```python
from build123d import *

# Parameters (mm, degrees)
SKETCH_1_W          = 50
SKETCH_1_H          = 50
SKETCH_1_W_2        = 44
SKETCH_1_H_2        = 44
EXTRUDE_2_DEPTH     = 190
SKETCH_5_R          = 6.5
CUT_EXTRUDE_1_DEPTH = 130


with BuildPart() as part:
    # 草图1 → 凸台-拉伸2 (new body)
    with BuildSketch(Plane.XY):
        with Locations((25, -25)):
            Rectangle(SKETCH_1_W, SKETCH_1_H)
        with Locations((25, -25)):
            Rectangle(SKETCH_1_W_2, SKETCH_1_H_2, mode=Mode.SUBTRACT)
    extrude(amount=EXTRUDE_2_DEPTH)

    # 草图5 → 切除-拉伸1 (cut)
    with BuildSketch(Plane(origin=(50, 0, 0), x_dir=(0, 0, -1), z_dir=(1, 0, 0))):
        with Locations(Location((-105, -25, 0), (0, 0, 90))):
            Circle(SKETCH_5_R)
        with Locations((-324.839370649, -25)):
            Circle(SKETCH_5_R)
    extrude(amount=-CUT_EXTRUDE_1_DEPTH, mode=Mode.SUBTRACT)


solid = part.part
```
CAD build for the part. Positions are in the model's coordinates, mm. A direction names the side the tool comes from. Round coordinates to 2 decimals unless told otherwise and drop trailing zeros. Order: outer loops, then holes, each group sorted by start corner. A loop starts at its lowest first (then second) coordinate and runs counter-clockwise, first axis right, second up.
Item 1: Saw through at D-D on z = 131. Write the cut outline in (x, y), then the cut area to 3 significant figures.
Item 2: Pin check, flat tip, straight feed: pin 1 (10.5 mm diameter, centred on y = -25, z = 105, fed in from +X). Stop position of the tip, or through.
Item 3: Saw through at C-C on y = -39.5. Write the cut outline in (x, z), then the cut area to 3 significant figures.
Item 4: Saw through at A-A on z = 105. Write the cut outline in (x, y), then the cut area to 3 significant figures.
Item 5: Saw through at B-B on x = 35. Write the cut outline in (y, z).
Item 6: Mould opens along Z. For faces 3 (the face through (1.521, -26.409, 98.655)), 4 (the face through (25, -3, 94)), 5 (the face through (2.7, -24.9, 0)), 6 (the face through (48.521, -26.409, 98.655)) say: pulls with the +Z half, pulls with the -Z half, needs draft (parallel to the pull), parting line crosses it, or undercut.
Item 7: Probe line 1 along X through (y, z) = (-37, 43.5); line 2 along Z through (x, y) = (48.8, -25); line 3 along Y through (x, z) = (24, 166). List the from-to ranges inside material, lowest first.
Item 8: Tool access for faces 1 (the face through (25, -50, 94)), 2 (the face through (3, -25, 94)): list every direction of +Z, -Z, +X, -X, +Y, -Y with a clear straight run to the whole face (end or side of a thin tool).
Reported:
1. outline: (0, -50) - (50, -50) - (50, 0) - (0, 0) - close; hole (3, -47) - (47, -47) - (47, -3) - (3, -3) - close
1. area: 564 mm2
2. pin 1: passes through
3. outline: (0, 0) - (3, 0) - (3, 190) - (0, 190) - close; (47, 0) - (50, 0) - (50, 190) - (47, 190) - close
3. area: 1,140 mm2
4. outline: (0, -50) - (50, -50) - (50, -31.5) - (47, -31.5) - (47, -47) - (3, -47) - (3, -31.5) - (0, -31.5) - close; (0, -18.5) - (3, -18.5) - (3, -3) - (47, -3) - (47, -18.5) - (50, -18.5) - (50, 0) - (0, 0) - close
4. area: 486 mm2
5. outline: (-50, 0) - (-47, 0) - (-47, 190) - (-50, 190) - close; (-3, 0) - (0, 0) - (0, 190) - (-3, 190) - close
6. face 3: undercut
6. face 4: needs draft
6. face 5: pulls with the -Z half
6. face 6: undercut
7. line 1: x = 0 to 3, 47 to 50
7. line 2: z = 0 to 98.5, 111.5 to 190
7. line 3: y = -50 to -47, -3 to 0
8. face 1: +Z, -Z, +X, -X, -Y
8. face 2: +Z, -Z
